CAD build for the part. Positions are in the model's coordinates, mm. A direction names the side the tool comes from. Round coordinates to 2 decimals unless told otherwise and drop trailing zeros. Write each loop counter-clockwise with the first axis right and the second up, starting at its lowest first coordinate (ties: lowest second). Pieces come first, ordered by that corner, then holes. Notation, with made-up numbers: (11, 15.5) - (59, 15.5) arc R25 ccw to (59, 39.5) - close; hole circle Ø7 at (-20, 20). An arc over 180 degrees is marked (long way). Put each result on its own line as item: value. Start each with the question number.
Item 1: 3-axis set-ups, long thin cutter, end or side, ignore diameter. For faces 5 (the flat face through (15, 39, -1)), 6 (the cylindrical face through (7.142, 37.096, -8.238)): which of +Z, -Z, +X, -X, +Y, -Y reach the whole face in a straight line?
Item 2: Drill centre lines: line 1 (Z direction, x = 4.5, y = -16); line 2 (Z direction, x = 6.75, y = 16.5); line 3 (Y direction, x = -9, z = 0). Where is each one in solid material? Low to high. Write a range as from..to.
Item 3: Cut at D-D (y = 14). Count the separate pieces of the cut face and the enclosed holes in it, and give its area (3 significant figures).
Item 4: Pin check, flat tips, straight feed: pin 1 Ø1 at (x, z) = (-8.5, -1) entering from +Y; pin 2 Ø9 at (y, z) = (12.29, 45.88) entering from +X; pin 3 Ø1 at (x, z) = (-1, -18) entering from +Y; pin 4 Ø1 at (x, z) = (-1, -36) entering from +Y. Stop position of each tip, or through.
Item 5: Mould opens along Y. For faces 1 (the flat face through (-0.5, 17, -26)), 2 (the cylindrical face through (0.21, 12.052, 40.387)), 3 (the cylindrical face through (0.2, -50.59, 32.26)), 4 (the flat face through (-15, -14, 27)) say: released by +Y, released by -Y, zero draft, split by the parting line, or undercut.
Item 6: Cut at A-A (z = 0). Give the cut face in (x, y), and give its area (3 significant figures).
Item 7: Cut at C-C (x = -10.5). Give the cut face in (y, z).
```python
from build123d import *

# Parameters (mm, degrees)
CHAMFER_1_SIZE           = 1
HOLE_WIZARD_M10_1_D      = 11
PATTERN_CIRCULAR_1_COUNT = 6


with BuildPart() as part:
    # 草图1 → 旋转1 (revolve)
    with BuildSketch(Plane(origin=(0, 0, 0), x_dir=(1, 0, 0), z_dir=(0, 1, 0)), mode=Mode.PRIVATE) as revolve_1_sk:
        Polygon((-15, 60), (15, 60), (15, 38), (-0.5, 38), (-0.5, 30.25), (-15, 30.25), align=None)
    revolve(revolve_1_sk.sketch.rotate(Axis((-222.715084562, 0, 0), (1, 0, 0)), 180), axis=Axis((-222.715084562, 0, 0), (1, 0, 0)))

    # 倒角1
    chamfer_1_edges = [part.edges().sort_by_distance(p)[0] for p in [
        (15, 0, -60),
        (-15, 0, -60),
    ]]
    chamfer(chamfer_1_edges, length=CHAMFER_1_SIZE)

    # M10 间隙孔1 (through all)
    with Locations(Plane.ZY.offset(15)):
        with Locations((33.587572106, -33.587572106)):
            hole_wizard_m10_1 = Hole(HOLE_WIZARD_M10_1_D / 2)

    # 阵列(圆周)1: M10 间隙孔1 ×6 about axis
    pattern_circular_1_axis = Axis((0, 0, 0), (1, 0, 0))
    for i in range(1, PATTERN_CIRCULAR_1_COUNT):
        add(hole_wizard_m10_1.rotate(pattern_circular_1_axis, i * 360 / PATTERN_CIRCULAR_1_COUNT), mode=Mode.SUBTRACT)


solid = part.part
```
Output values:
1. face 5: +Z, -Z, +X, +Y, -Y
1. face 6: +X
2. line 1: -57.83..-49.95, -41.82..-34.47, 34.47..57.83
2. line 2: -57.69..-34.23, 34.23..42.34, 49.43..57.69
2. line 3: -60..-30.25, 30.25..60
3. separate pieces: 3
3. enclosed holes: 0
3. area: 1,310 mm2
4. pin 1: y = 60
4. pin 2: through
4. pin 3: y = 57.39
4. pin 4: y = 48.37
5. face 1: undercut
5. face 2: undercut
5. face 3: split by the parting line
5. face 4: zero draft
6. outline: (-15, -59) - (-14, -60) - (14, -60) - (15, -59) - (15, -38) - (-0.5, -38) - (-0.5, -30.25) - (-15, -30.25) - close; (-15, 30.25) - (-0.5, 30.25) - (-0.5, 38) - (15, 38) - (15, 59) - (14, 60) - (-14, 60) - (-15, 59) - close
6. area: 1,540 mm2
7. outline: circle Ø120 at (0, 0); hole circle Ø11 at (-45.88, -12.29); hole circle Ø11 at (-33.59, 33.59); hole circle Ø60.5 at (0, 0); hole circle Ø11 at (-12.29, -45.88); hole circle Ø11 at (12.29, 45.88); hole circle Ø11 at (33.59, -33.59); hole circle Ø11 at (45.88, 12.29)
